Model file for the job. Use its own axes, mm. Face numbers are marked on the shaded views. A direction names the side the tool comes from. Coordinates: 2 decimals unless noted, no trailing zeros. Write each loop counter-clockwise with the first axis right and the second up, starting at its lowest first coordinate (ties: lowest second). Pieces come first, ordered by that corner, then holes. Notation, with made-up numbers: M 15.25,25.5 L 34.25,25.5 A21 cw 34.25,38.5 Z; hole C -20,-13 d8. An arc over 180 degrees is marked long. Put each result on its own line as item: value. Start each with the question number.
Q1. Cut at B-B (z = 11). Write the cut outline in (x, y).
Q2. Drill centre lines: line 1 along Y through (x, z) = (0, -14); line 2 along X through (y, z) = (10, -1.5); line 3 along Z through (x, y) = (-1.5, 10.75). Where is each one in solid material? Low to high.
Q3. Cut at C-C (x = 0). Write the cut outline in (y, z).
Q4. Which spindle directions (+Z, -Z, +X, -X, +Y, -Y) get a long thin tool onto all of the face, cutting with end or side? Do the marked faces 5 and 6. Say none if no direction does.
Q5. Cut at D-D (y = 6). Write the cut outline in (x, z).
Q6. Pull direction X, two halves, no side cores. Call the marked faces 1, 2, 3 and 4: pulls with the +X half, pulls with the -X half, needs draft (parallel to the pull), parting line crosses it, or undercut.
Q7. Cut at A-A (x = 6). Write the cut outline in (y, z).
Q8. Drop flat-ended pins along their axis: pin 1 (4 mm diameter, centred on x = -1, y = 10, fed in from +Z); pin 2 (2 mm diameter, centred on x = 5, z = 5, fed in from +Y); pin 3 (3 mm diameter, centred on y = 3, z = 13, fed in from +X). Give the stop position or say it passes through.
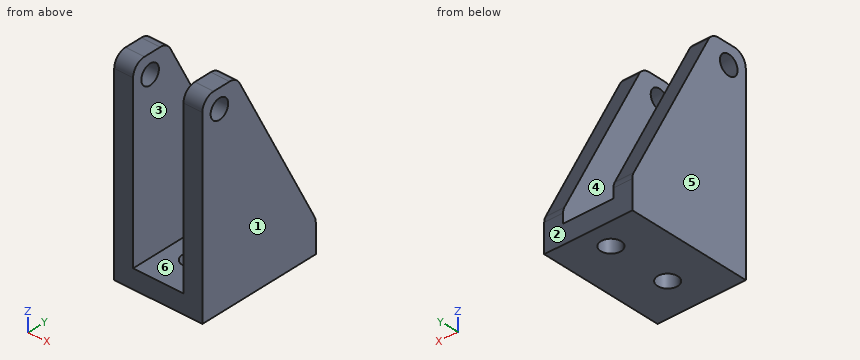
```python
from build123d import *

# Parameters (mm, degrees)
SKETCH_1_W          = 14
SKETCH_1_H          = 32
EXTRUDE_1_DEPTH     = 20
CUT_EXTRUDE_1_DEPTH = 20
SKETCH_3_W          = 8
SKETCH_3_H          = 29
CUT_EXTRUDE_2_DEPTH = 20
FILLET_2_R          = 2
SKETCH_4_R          = 1.55
CUT_EXTRUDE_3_DEPTH = 20
SKETCH_5_R          = 1.6
CUT_EXTRUDE_4_DEPTH = 20


with BuildPart() as part:
    # 草图1 → 凸台-拉伸1 (new body)
    with BuildSketch(Plane(origin=(0, 0, 0), x_dir=(1, 0, 0), z_dir=(0, 1, 0))):
        Rectangle(SKETCH_1_W, SKETCH_1_H)
    extrude(amount=EXTRUDE_1_DEPTH)

    # 草图2 → 切除-拉伸1 (cut)
    with BuildSketch(Plane(origin=(7, 0, 0), x_dir=(0, 0, -1), z_dir=(1, 0, 0))):
        Polygon((-16, 6), (11, 20), (-16, 20), align=None)
    extrude(amount=-CUT_EXTRUDE_1_DEPTH, mode=Mode.SUBTRACT)

    # 草图3 → 切除-拉伸2 (cut)
    with BuildSketch(Plane.XZ):
        with Locations((0, 1.5)):
            Rectangle(SKETCH_3_W, SKETCH_3_H)
    extrude(amount=-CUT_EXTRUDE_2_DEPTH, mode=Mode.SUBTRACT)

    # 圆角2
    fillet_2_edges = [part.edges().sort_by_distance(p)[0] for p in [
        (-5.5, 20, -11),
        (-5.5, 6, 16),
        (5.5, 6, 16),
        (5.5, 20, -11),
        (5.5, 0, 16),
        (-5.5, 0, 16),
    ]]
    fillet(fillet_2_edges, radius=FILLET_2_R)

    # 草图4 → 切除-拉伸3 (cut)
    with BuildSketch(Plane.ZY.offset(7)):
        with Locations((13, 3)):
            Circle(SKETCH_4_R)
    extrude(amount=-CUT_EXTRUDE_3_DEPTH, mode=Mode.SUBTRACT)

    # 草图5 → 切除-拉伸4 (cut)
    with BuildSketch(Plane.XY.offset(-13)):
        with Locations((0, 16)):
            Circle(SKETCH_5_R)
        with Locations((0, 6)):
            Circle(SKETCH_5_R)
    extrude(amount=-CUT_EXTRUDE_4_DEPTH, mode=Mode.SUBTRACT)


solid = part.part
```
Computed values:
1. outline: M -7,0 L -4,0 L -4,8.59 L -7,8.59 Z; M 4,0 L 7,0 L 7,8.59 L 4,8.59 Z
2. line 1: 0 to 4.4, 7.6 to 14.4, 17.6 to 20
2. line 2: -7 to -4, 4 to 7
2. line 3: -16 to -13
3. outline: M 0,-16 L 4.4,-16 L 4.4,-13 L 0,-13 Z; M 7.6,-16 L 14.4,-16 L 14.4,-13 L 7.6,-13 Z; M 17.6,-16 L 20,-16 L 20,-13 L 17.6,-13 Z
4. face 5: +Z, -Z, -X, +Y, -Y
4. face 6: +Z, +Y, -Y
5. outline: M -7,-16 L -1.6,-16 L -1.6,-13 L -4,-13 L -4,15.59 L -7,15.59 Z; M 1.6,-16 L 7,-16 L 7,15.59 L 4,15.59 L 4,-13 L 1.6,-13 Z
6. face 1: pulls with the +X half
6. face 2: needs draft
6. face 3: undercut
6. face 4: undercut
7. outline: M 0,-16 L 20,-16 L 20,-11.49 A2 ccw 19.78,-10.57 L 6.56,14.92 A2 ccw 4.78,16 L 2,16 A2 ccw 0,14 Z; hole C 3,13 d3.1
8. pin 1: z = -13
8. pin 2: y = 12.22
8. pin 3: through
